from build123d import *

# Parameters (mm, degrees)
PIVOT_BOSS_SKETCH_R   = 27
PIVOT_BOSS_SKETCH_R_2 = 11.5
PIVOT_BOSS_DEPTH      = 38
MOUNTING_PLATE_DEPTH  = 25
ARM_BLOCK_DEPTH       = 60
PIVOT_BORE_SKETCH_R   = 12.5
PIVOT_BORE_25_DEPTH   = 60
CLAMP_TAB_SKETCH_R    = 6
CLAMP_TAB_DEPTH       = 10


with BuildPart() as part:
    # Pivot Boss Sketch → Pivot Boss (new body)
    with BuildSketch(Plane.XY):
        Circle(PIVOT_BOSS_SKETCH_R)
        Circle(PIVOT_BOSS_SKETCH_R_2, mode=Mode.SUBTRACT)
    extrude(amount=PIVOT_BOSS_DEPTH)

    # Mounting Plate Sketch → Mounting Plate (add)
    with BuildSketch(Plane.XY):
        with BuildLine():
            Line((-8.1, 25.756358438), (82.9, 54.374534481))
            ThreePointArc((82.9, 54.374534481), (157, 0), (82.9, -54.374534481))
            Line((82.9, -54.374534481), (-8.1, -25.756358438))
            ThreePointArc((-8.1, -25.756358438), (27, 0), (-8.1, 25.756358438))
        make_face()
    extrude(amount=MOUNTING_PLATE_DEPTH)

    # Arm Block Sketch → Arm Block (add)
    with BuildSketch(Plane.XY.offset(25)):
        with BuildLine():
            Line((60, 27), (115, 27))
            Line((115, 27), (115, -27))
            Line((115, -27), (60, -27))
            ThreePointArc((60, -27), (33, 0), (60, 27))
        make_face()
    extrude(amount=ARM_BLOCK_DEPTH)

    # Pivot Bore Sketch → Pivot Bore Ø25 (cut)
    with BuildSketch(Plane.XY.offset(85)):
        with Locations((60, 0)):
            Circle(PIVOT_BORE_SKETCH_R)
    extrude(amount=-PIVOT_BORE_25_DEPTH, mode=Mode.SUBTRACT)

    # Clamp Tab Sketch → Clamp Tab (add)
    with BuildSketch(Plane.XZ.offset(27)):
        with BuildLine():
            Line((90, 63), (90, 25))
            Line((90, 25), (110, 25))
            Line((110, 25), (110, 63))
            ThreePointArc((110, 63), (100, 73), (90, 63))
        make_face()
        with Locations(Location((100, 63, 0), (0, 0, 270))):
            Circle(CLAMP_TAB_SKETCH_R, mode=Mode.SUBTRACT)
    clamp_tab = extrude(amount=CLAMP_TAB_DEPTH)

    # Clamp Tab Mirror: Clamp Tab across plane
    add(clamp_tab.mirror(Plane.ZX))


solid = part.part
Verification items for the finished model (mm, model axes). A direction names the side the tool comes from. Give positions to 0.01 mm unless a question says otherwise; leave off trailing zeros. Loops run counter-clockwise (first coordinate to the right, second up) from the corner with the lowest first, then second, coordinate; pieces in that order, holes last.
1) Draft check along X on faces 1 (the cylindrical face through (156.98, 1.5, 12.32)), 2 (the flat face through (100, 37, 44)), 3 (the cylindrical face through (-26.974, 1.187, 22.956)). Enter one of: pulls with the +X half, pulls with the -X half, needs draft (parallel to the pull), parting line crosses it, or undercut.
2) Sectioned sample at A-A, the plane y = 0. Enter the section's corners in (x, z), then the cut area to 3 significant figures.
3) Sectioned sample at D-D, the plane x = 100. Enter the section's corners in (y, z), then the cut area to 3 significant figures.
4) Depth check by flat-ended pin: pin 1 Ø3 at (y, z) = (32.5, 39) entering from -X; pin 2 Ø6 at (x, y) = (38, 17.5) entering from +Z; pin 3 Ø6 at (x, z) = (2, 38.5) entering from -Y; pin 4 Ø6 at (x, z) = (105.5, 68.5) entering from +Y. Enter the tip coordinate at first touch or a pass-through.
5) Set-up check for faces 4 (the cylindrical face through (50.08, -7.606, 55.42)), 5 (the flat face through (100, -27, 63)), 6 (the flat face through (90, 32, 44)): record each of +Z, -Z, +X, -X, +Y, -Y from which the full face is reachable in a straight line by a thin tool's end or side.
6) Sectioned sample at B-B, the plane z = 48.5. Enter the section's corners in (x, y), then the cut area to 3 significant figures.
7) Thickness scan on line 1 along X through (y, z) = (-31.75, 63); line 2 along Y through (x, z) = (1, 29); line 3 along Y through (x, z) = (76, 74). Record the ranges inside material, lowest first.
8) Sectioned sample at C-C, the plane x = 0. Enter the section's corners in (y, z), then the cut area to 3 significant figures.
Answers:
1. face 1: parting line crosses it
1. face 2: needs draft
1. face 3: undercut
2. outline: (-27, 0) - (-11.5, 0) - (-11.5, 38) - (-27, 38) - close; (11.5, 0) - (157, 0) - (157, 25) - (115, 25) - (115, 85) - (72.5, 85) - (72.5, 25) - (47.5, 25) - (47.5, 85) - (33, 85) - (33, 25) - (27, 25) - (27, 38) - (11.5, 38) - close
2. area: 7,850 mm2
3. outline: (-57, 0) - (57, 0) - (57, 25) - (37, 25) - (37, 57) - (27, 57) - (27, 69) - (37, 69) - (37, 73) - (27, 73) - (27, 85) - (-27, 85) - (-27, 73) - (-37, 73) - (-37, 69) - (-27, 69) - (-27, 57) - (-37, 57) - (-37, 25) - (-57, 25) - close
3. area: 6,810 mm2
4. pin 1: stops at x = 90
4. pin 2: stops at z = 85
4. pin 3: stops at y = -27
4. pin 4: stops at y = 37
5. face 4: +Z
5. face 5: -Y
5. face 6: +Z, -X, +Y
6. outline: (60, -27) - (90, -27) - (90, -37) - (110, -37) - (110, -27) - (115, -27) - (115, 27) - (110, 27) - (110, 37) - (90, 37) - (90, 27) - (60, 27) arc R27 ccw to start; hole circle Ø25 at (60, 0)
6. area: 4,020 mm2
7. line 1: x = 90 to 94, 106 to 110
7. line 2: y = -26.98 to -11.46, 11.46 to 26.98
7. line 3: y = -27 to 27
8. outline: (-28.3, 0) - (-11.5, 0) - (-11.5, 38) - (-27, 38) - (-27, 25) - (-28.3, 25) - close; (11.5, 0) - (28.3, 0) - (28.3, 25) - (27, 25) - (27, 38) - (11.5, 38) - close
8. area: 1,240 mm2
